from build123d import *

# Parameters (mm, degrees)
EXTRUDE_390_DEPTH = 6.4
FILLET_1290_R     = 0.4


with BuildPart() as part:
    # 草图1 → Extrude 390 (new body)
    with BuildSketch(Plane(origin=(0, 0, 0), x_dir=(0, 0, -1), z_dir=(1, 0, 0))):
        Polygon((8, 4.618802154), (8, -4.618802154), (0, -9.237604307), (-8, -4.618802154), (-8, 4.618802154), (0, 9.237604307), align=None)
    extrude(amount=EXTRUDE_390_DEPTH)

    # 草图2 → 凸台-旋转1 (revolve)
    with BuildSketch(Plane.XY, mode=Mode.PRIVATE) as revolve_1_sk:
        Polygon((0, 0), (31.4, 0), (31.4, 3.701), (31.4, 5), (0, 5), align=None)
    revolve(revolve_1_sk.sketch.rotate(Axis((0, 0, 0), (1, 0, 0)), 90), axis=Axis((0, 0, 0), (1, 0, 0)))

    # 草图3 → 切除-旋转1 (revolve, cut)
    with BuildSketch(Plane.XY):
        Polygon((0, 8), (3.601282526, 14.237604307), (3.601282526, 19.237604307), (-10, 19.237604307), (-10, 8), align=None)
    revolve(axis=Axis((0, 0, 0), (1, 0, 0)), mode=Mode.SUBTRACT)

    # 草图4 → 切除-旋转3 (revolve, cut)
    with BuildSketch(Plane.XY, mode=Mode.PRIVATE) as cut_revolve_3_sk:
        Polygon((6.4, 7.315), (5.8, 7.661410162), (5.8, 9.237604307), (6.4, 9.237604307), align=None)
    revolve(cut_revolve_3_sk.sketch.rotate(Axis((0, 0, 0), (1, 0, 0)), 90), axis=Axis((0, 0, 0), (1, 0, 0)), mode=Mode.SUBTRACT)

    # Fillet 1290
    fillet_1290_edges = [part.edges().sort_by_distance(p)[0] for p in [
        (6.4, 0, -5),
    ]]
    fillet(fillet_1290_edges, radius=FILLET_1290_R)

    # 草图6 → 切除-旋转4 (revolve, cut)
    with BuildSketch(Plane.XY, mode=Mode.PRIVATE) as cut_revolve_4_sk:
        Polygon((30.65, 5), (32.15, 5), (31.4, 3.700961894), align=None)
    revolve(cut_revolve_4_sk.sketch.rotate(Axis((0, 0, 0), (1, 0, 0)), 90), axis=Axis((0, 0, 0), (1, 0, 0)), mode=Mode.SUBTRACT)


solid = part.part
Here's how the part is built. I have some questions about the finished solid (model axes, mm). A direction names the side the tool comes from. Round coordinates to 2 decimals unless told otherwise and drop trailing zeros. Loops run counter-clockwise (first coordinate to the right, second up) from the corner with the lowest first, then second, coordinate; pieces in that order, holes last. Notation, with made-up numbers: (-13, -15.75) - (-4, -15.75) arc R33 cw to (-4, 13.25) - close; hole circle Ø8 at (-28.5, 57.25). An arc over 180 degrees is marked (long way). One line per question, with ' | ' between items. Start each with the question number.
Q1. For faces 1 (the conical face through (0.174, -4.133, 7.199)), 2 (the flat face through (5.8, 7.5, 2.4)), which set-ups out of +Z, -Z, +X, -X, +Y, -Y let a thin tool reach every point of the face, with its end or its side?
Q2. I want a section at A-A (x = 22.5). Write out the boundary of the cut face in (y, z), then the cut area to 3 significant figures.
Q3. Will these pins go through, and if not, where does the flat tip stop? pin 1 (1 mm diameter, centred on x = 23, y = 1.5, fed in from +Z); pin 2 (1 mm diameter, centred on x = 18.5, y = -3, fed in from -Z); pin 3 (6 mm diameter, centred on x = 18, z = 3, fed in from -Y).
Q4. Please list where these lines run through material, in increasing order: line 1 (X direction, y = 6, z = -3.25); line 2 (Z direction, x = 17, y = -0.25); line 3 (X direction, y = -5.5, z = 5.75). Write a range as [from, to].
Response values:
1) face 1: +Z, -X, -Y | face 2: +X
2) outline: circle Ø10 at (0, 0) | area: 78.5 mm²
3) pin 1: stops at z = 4.9 | pin 2: stops at z = -4.33 | pin 3: stops at y = -5
4) line 1: x = [0, 6.4] | line 2: z = [-4.99, 4.99] | line 3: x = [0, 5.8]
